Can you work these out from the model? Positions are in its coordinate system, mm. A direction names the side the tool comes from. Give positions to 0.01 mm unless a question says otherwise; leave off trailing zeros. Write each loop counter-clockwise with the first axis right and the second up, starting at its lowest first coordinate (ties: lowest second). Pieces come first, ordered by that corner, then holes.
```python
from build123d import *

# Parameters (mm, degrees)
BASE_SHANK_PROFILE_25_2_R  = 12.5
BASE_SHANK_25_2_DEPTH      = 25.2
TAPER_START_PROFILE_25_2_R = 12.5
TAPER_END_PROFILE_20_2_R   = 10
THROUGH_SLOT_PROFILE_W     = 7
THROUGH_SLOT_PROFILE_H     = 24
THROUGH_SLOT_DEPTH         = 17.6


with BuildPart() as part:
    # Base Shank Profile Ø25.2 → Base Shank Ø25.2 (new body)
    with BuildSketch(Plane(origin=(0, 0, 0), x_dir=(1, 0, 0), z_dir=(0, 1, 0))):
        with Locations(Location((0, 0, 0), (0, 0, 270))):
            Circle(BASE_SHANK_PROFILE_25_2_R)
    extrude(amount=BASE_SHANK_25_2_DEPTH)

    # Taper Start Profile Ø25.2 → Tapered Rod Loft section 0
    with BuildSketch(Plane(origin=(0, 25.2, 0), x_dir=(1, 0, 0), z_dir=(0, 1, 0))):
        Circle(TAPER_START_PROFILE_25_2_R)
    # Taper End Profile Ø20.2 → Tapered Rod Loft section 1
    with BuildSketch(Plane(origin=(0, 117.2, 0), x_dir=(1, 0, 0), z_dir=(0, 1, 0))):
        Circle(TAPER_END_PROFILE_20_2_R)
    loft()

    # Through Slot Profile → Through Slot (cut, symmetric)
    with BuildSketch(Plane.XY):
        with Locations((0, 70.2)):
            Rectangle(THROUGH_SLOT_PROFILE_W, THROUGH_SLOT_PROFILE_H)
    extrude(amount=THROUGH_SLOT_DEPTH, both=True, mode=Mode.SUBTRACT)


solid = part.part
```
1) Please list where these lines run through material, in increasing order: L1, parallel to Y at x = 2.75, z = 6; L2, parallel to X at y = 66, z = -9.75; L3, parallel to X at y = 64, z = 4.5.
Values follow:
L1: y = 0 to 58.2, 82.2 to 117.2
L2: x = -5.89 to -3.5, 3.5 to 5.89
L3: x = -10.52 to -3.5, 3.5 to 10.52
2) For faces 1 (the face through (3.5, 70, 0)), 2 (the face through (3.755, 12.424, 11.923)), which set-ups out of +Z, -Z, +X, -X, +Y, -Y let a thin tool reach every point of the face, with its end or its side?
Values follow:
face 1: +Z, -Z
face 2: +Y, -Y
3) Suppose I cut it at B-B on y = 8.5. Write out the boundary of the cut face in (x, z).
Values follow:
outline: circle Ø25 at (0, 0)
4) Suppose I cut it at C-C on y = 74. Write out the boundary of the cut face in (x, z).
Values follow:
outline: (-3.5, -10.61) - (-3.5, 10.61) arc R11.17 ccw to start; (3.5, -10.61) arc R11.17 ccw to (3.5, 10.61) - close
5) Suppose I cut it at D-D on y = 37. Write out the boundary of the cut face in (x, z), plus the area to 3 significant figures.
Values follow:
outline: circle Ø24.36 at (0, 0)
area: 466 mm2
6) For pin 1 Ø5 at (x, y) = (-3.5, 23.5) entering from -Z; pin 2 Ø4 at (x, y) = (8, 55) entering from +Z; pin 3 Ø3 at (y, z) = (81.5, -2) entering from -X, each with a flat end and sliding along its axis, tell me the tip position at first contact or that it passes through.
Values follow:
pin 1: stops at z = -12.46
pin 2: stops at z = 10.03
pin 3: stops at x = -10.97
7) Suppose I cut it at A-A on x = 0. Write out the boundary of the cut face in (y, z).
Values follow:
outline: (0, -12.5) - (25.2, -12.5) - (58.2, -11.6) - (58.2, 11.6) - (25.2, 12.5) - (0, 12.5) - close; (82.2, -10.95) - (117.2, -10) - (117.2, 10) - (82.2, 10.95) - close
8) If we mould it in two halves opening along X, with no side actions, what happens to faces 3 (the face through (0, 0, 0)), 4 (the face through (10.714, 71.844, -3.374)), 5 (the face through (0, 82.2, 0))? For each: +X half, -X half, draft (parallel to the pull), parting line (faces both ways), or undercut.
Values follow:
face 3: draft
face 4: parting line
face 5: undercut
